The listing builds one solid part. Answer for the finished solid, in the listing's coordinates (mm). Coordinates: 2 decimals unless noted, no trailing zeros. Order: outer loops, then holes, each group sorted by start corner. A loop starts at its lowest first (then second) coordinate and runs counter-clockwise, first axis right, second up. Notation, with made-up numbers: (67.25, -5) - (114.25, -5) arc R20 ccw to (114.25, 20) - close; hole circle Ø8 at (43.25, -4.5). An arc over 180 degrees is marked (long way). One line per item, written item: value. Start each with the question number.
```python
from build123d import *
from OCP.BRepFilletAPI import BRepFilletAPI_MakeChamfer

# Parameters (mm, degrees)
SKETCH_1_R            = 6.5
SKETCH_1_R_2          = 4
EXTRUDE_1_DEPTH       = 44
HOLE_WIZARD_4_0_4_1_D = 4
CHAMFER_1_SIZE        = 0.5
CHAMFER_2_SIZE        = 1
CHAMFER_2_SIZE2       = 1.732050808


with BuildPart() as part:
    # 草图1 → 凸台-拉伸1 (new body)
    with BuildSketch(Plane(origin=(0, 0, 0), x_dir=(1, 0, 0), z_dir=(0, 1, 0))):
        with Locations(Location((0, 0, 0), (0, 0, 270))):
            Circle(SKETCH_1_R)
        with Locations(Location((0, 0, 0), (0, 0, 270))):
            Circle(SKETCH_1_R_2, mode=Mode.SUBTRACT)
    extrude(amount=EXTRUDE_1_DEPTH)

    # Ø4.0 (4) 直径孔1 (through all)
    with Locations(Plane(origin=(6.5, 6, 0), x_dir=(0, 0, 1), z_dir=(1, 0, 0))):
        with Locations((0, 0)):
            Hole(HOLE_WIZARD_4_0_4_1_D / 2)

    # 倒角1
    chamfer_1_edges = [part.edges().sort_by_distance(p)[0] for p in [
        (0, 0, -6.5),
        (0, 44, -6.5),
    ]]
    chamfer(chamfer_1_edges, length=CHAMFER_1_SIZE)

    # 倒角2: one chamfer whose edges measure the first distance from different faces: ONE call of the kernel's chamfer builder (chamfer() names one face for all edges)
    chamfer_2_edges_1 = [part.edges().sort_by_distance(p)[0] for p in [
        (0, 0, -4),
    ]]
    chamfer_2_side_1 = [part.faces().sort_by_distance(p)[0] for p in [
        (0, 0, -5.830294373),
    ]]
    chamfer_2_edges_2 = [part.edges().sort_by_distance(p)[0] for p in [
        (0, 44, -4),
    ]]
    chamfer_2_side_2 = [part.faces().sort_by_distance(p)[0] for p in [
        (0, 44, -5.830294373),
    ]]
    chamfer_2 = BRepFilletAPI_MakeChamfer(part.part.solid().wrapped)
    for e in chamfer_2_edges_1:
        chamfer_2.Add(CHAMFER_2_SIZE, CHAMFER_2_SIZE2, e.wrapped, chamfer_2_side_1[0].wrapped)  # the first distance lies on this face
    for e in chamfer_2_edges_2:
        chamfer_2.Add(CHAMFER_2_SIZE, CHAMFER_2_SIZE2, e.wrapped, chamfer_2_side_2[0].wrapped)  # the first distance lies on this face
    add(Compound.cast(chamfer_2.Shape()), mode=Mode.REPLACE)


solid = part.part
```
(1) For a pull along X with two mould halves and no side action, classify faces 1 (the face through (4, 44, -4)), 2 (the face through (1.95, 21.7, 6.2)), 3 (the face through (-3.905, 21.716, -0.867)) as pulls with the +X half, pulls with the -X half, needs draft (parallel to the pull), parting line crosses it, or undercut.
(2) The part is cut by section D-D on y = 27. Determine the outline of the cut face in (x, z), plus the area to 3 significant figures.
(3) The part is cut by section A-A on x = 0. Determine the outline of the cut face in (y, z), plus the area to 3 significant figures.
(4) Consider probe 1 along X at (y, z) = (34.5, 0.25); probe 2 along Y at (x, z) = (-5.1, 0); probe 3 along Z at (x, y) = (-5.5, 31). Determine where each line is inside the solid, lowest interval first.
(5) The part is cut by section B-B on z = 0. Determine the outline of the cut face in (x, y), plus the area to 3 significant figures.
(6) The part is cut by section C-C on y = 6. Determine the outline of the cut face in (x, z), plus the area to 3 significant figures.
(7) Flat-ended cylindrical pins translate along their axes: pin 1 Ø5 at (x, z) = (-4.5, 2) entering from +Y; pin 2 Ø7 at (x, z) = (0, 0) entering from -Y; pin 3 Ø1 at (x, y) = (-1, 14.5) entering from +Z; pin 4 Ø2 at (y, z) = (17, 4.5) entering from -X. Find the tip coordinate at first contact, or state that the pin passes through.
Completed:
1. face 1: needs draft
1. face 2: parting line crosses it
1. face 3: undercut
2. outline: circle Ø13 at (0, 0); hole circle Ø8 at (0, 0)
2. area: 82.5 mm2
3. outline: (0, -6) - (0.5, -6.5) - (43.5, -6.5) - (44, -6) - (44, -5) - (42.27, -4) - (1.73, -4) - (0, -5) - close; (0, 5) - (1.73, 4) - (42.27, 4) - (44, 5) - (44, 6) - (43.5, 6.5) - (0.5, 6.5) - (0, 6) - close
3. area: 216 mm2
4. probe 1: x = -6.5 to -3.99, 3.99 to 6.5
4. probe 2: y = 0 to 4, 8 to 44
4. probe 3: z = -3.46 to 3.46
5. outline: (-6.5, 0.5) - (-6, 0) - (-5, 0) - (-4, 1.73) - (-4, 4) - (-6.5, 4) - close; (-6.5, 8) - (-4, 8) - (-4, 42.27) - (-5, 44) - (-6, 44) - (-6.5, 43.5) - close; (4, 1.73) - (5, 0) - (6, 0) - (6.5, 0.5) - (6.5, 4) - (4, 4) - close; (4, 8) - (6.5, 8) - (6.5, 43.5) - (6, 44) - (5, 44) - (4, 42.27) - close
5. area: 196 mm2
6. outline: (-6.18, -2) arc R6.5 ccw to (6.18, -2) - (3.46, -2) arc R4 cw to (-3.46, -2) - close; (-6.18, 2) - (-3.46, 2) arc R4 cw to (3.46, 2) - (6.18, 2) arc R6.5 ccw to start
6. area: 61.9 mm2
7. pin 1: stops at y = 44
7. pin 2: passes through
7. pin 3: stops at z = 6.48
7. pin 4: stops at x = -5.48
